Design review of the part built by this model. Coordinates are the model's own, in mm. Coordinates: 2 decimals unless noted, no trailing zeros. Write each loop counter-clockwise with the first axis right and the second up, starting at its lowest first coordinate (ties: lowest second). Pieces come first, ordered by that corner, then holes.
Q1. To check wall thickness, follow probe 1 along X at (y, z) = (0, 2.5); probe 2 along Y at (x, z) = (-40, 3); probe 3 along X at (y, z) = (-11.5, 1). State the ranges of each line that lie inside material, in increasing order.
Q2. Add section C-C, the plane x = -40. Give the boundary of the cut face in (y, z) (3 decimals).
Q3. Clearance check with flat-ended pins moving along their axes: pin 1 Ø12 at (x, y) = (-3.5, 9.5) entering from -Z; pin 2 Ø5.5 at (x, y) = (-40, 0) entering from -Z. State where each tip first meets the part, or that it passes through.
Q4. Add section A-A, the plane y = 0. Give the boundary of the cut face in (x, z) (3 decimals), plus the area to 3 significant figures.
Q5. Add section B-B, the plane z = 4.5. Give the boundary of the cut face in (x, y).
from build123d import *

# Parameters (mm, degrees)
SKETCH1_W                   = 100
SKETCH1_H                   = 30
BOSS_EXTRUDE1_DEPTH         = 8
FILLET1_R                   = 5
M8_TAPPED_HOLE1_D           = 6.8
M8_TAPPED_HOLE1_CSINK_D     = 8.05
M8_TAPPED_HOLE1_CSINK_ANGLE = 90


with BuildPart() as part:
    # Sketch1 → Boss-Extrude1 (new body)
    with BuildSketch(Plane.XY):
        Rectangle(SKETCH1_W, SKETCH1_H)
    extrude(amount=BOSS_EXTRUDE1_DEPTH)

    # Fillet1
    fillet1_edges = [part.edges().sort_by_distance(p)[0] for p in [
        (50, -15, 4),
        (-50, -15, 4),
        (-50, 15, 4),
        (50, 15, 4),
    ]]
    fillet(fillet1_edges, radius=FILLET1_R)

    # M8 Tapped Hole1 (through all)
    with Locations(Plane.XY.offset(8)):
        with Locations((-40, 0), (40, 0)):
            CounterSinkHole(M8_TAPPED_HOLE1_D / 2, M8_TAPPED_HOLE1_CSINK_D / 2, counter_sink_angle=M8_TAPPED_HOLE1_CSINK_ANGLE)


solid = part.part
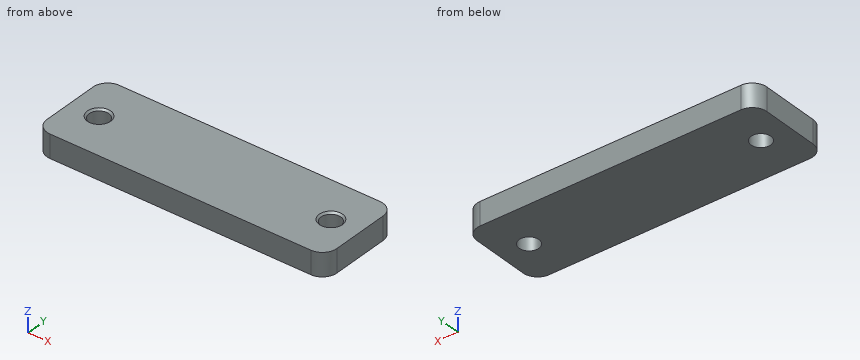
Here are the results:
1. probe 1: x = -50 to -43.4, -36.6 to 36.6, 43.4 to 50
1. probe 2: y = -15 to -3.4, 3.4 to 15
1. probe 3: x = -49.77 to 49.77
2. outline: (-15, 0) - (-3.4, 0) - (-3.4, 7.375) - (-4.025, 8) - (-15, 8) - close; (3.4, 0) - (15, 0) - (15, 8) - (4.025, 8) - (3.4, 7.375) - close
3. pin 1: stops at z = 0
3. pin 2: passes through
4. outline: (-50, 0) - (-43.4, 0) - (-43.4, 7.375) - (-44.025, 8) - (-50, 8) - close; (-36.6, 0) - (36.6, 0) - (36.6, 7.375) - (35.975, 8) - (-35.975, 8) - (-36.6, 7.375) - close; (43.4, 0) - (50, 0) - (50, 8) - (44.025, 8) - (43.4, 7.375) - close
4. area: 690 mm2
5. outline: (-50, -10) arc R5 ccw to (-45, -15) - (45, -15) arc R5 ccw to (50, -10) - (50, 10) arc R5 ccw to (45, 15) - (-45, 15) arc R5 ccw to (-50, 10) - close; hole circle Ø6.8 at (-40, 0); hole circle Ø6.8 at (40, 0)
